```python
from build123d import *

# Parameters (mm, degrees)
SKETCH_1_R      = 17.5
EXTRUDE_1_DEPTH = 31
SKETCH_2_R      = 15
EXTRUDE_2_DEPTH = 43
SKETCH_4_R      = 18.5
EXTRUDE_3_DEPTH = 4


with BuildPart() as part:
    # 草图1 → 凸台-拉伸1 (new body)
    with BuildSketch(Plane(origin=(0, 0, 0), x_dir=(0, 0, -1), z_dir=(1, 0, 0))):
        Circle(SKETCH_1_R)
    extrude(amount=EXTRUDE_1_DEPTH)

    # 草图2 → 凸台-拉伸2 (add)
    with BuildSketch(Plane.ZY):
        with Locations(Location((0, 0, 0), (0, 0, 180))):
            Circle(SKETCH_2_R)
    extrude(amount=EXTRUDE_2_DEPTH)

    # 草图4 → 凸台-拉伸3 (add)
    with BuildSketch(Plane(origin=(12, 0, 0), x_dir=(0, 0, -1), z_dir=(1, 0, 0))):
        Circle(SKETCH_4_R)
    extrude(amount=EXTRUDE_3_DEPTH)


solid = part.part
```
Can you work these out from the model? Positions are in its coordinate system, mm. A direction names the side the tool comes from. Round coordinates to 2 decimals unless told otherwise and drop trailing zeros. Loops run counter-clockwise (first coordinate to the right, second up) from the corner with the lowest first, then second, coordinate; pieces in that order, holes last.
Item 1: Will these pins go through, and if not, where does the flat tip stop? pin 1 Ø3 at (x, z) = (23, -1) entering from +Y; pin 2 Ø5 at (x, z) = (18, -2) entering from -Y; pin 3 Ø1.5 at (x, y) = (12.5, 11.5) entering from +Z; pin 4 Ø8 at (x, y) = (17.5, 1.5) entering from -Z.
Item 2: Which directions (+Z, -Z, +X, -X, +Y, -Y) give clear straight access to the entire face, cutting with the end or side of a thin tool? Please do faces 1 (the cylindrical face through (5.916, -10.648, 13.887)), 2 (the flat face through (16, -14, 11)), 3 (the cylindrical face through (13.97, -18.06, 4.01)).
Item 3: Suppose I cut it at C-C, the plane x = 13. Write out the boundary of the cut face in (y, z).
Item 4: Please list where these lines run through material, in increasing order: L1, parallel to X at y = 9, z = 16; L2, parallel to X at y = 9.5, z = -12; L3, parallel to Y at x = -36, z = -7.5.
Item 5: Suppose I cut it at D-D, the plane x = 24.5. Write out the boundary of the cut face in (y, z).
Item 6: Suppose I cut it at A-A, the plane z = 0. Write out the boundary of the cut face in (x, y).
Reported:
1. pin 1: stops at y = 17.5
1. pin 2: stops at y = -18.49
1. pin 3: stops at z = 15.06
1. pin 4: stops at z = -18.5
2. face 1: -X
2. face 2: +X
2. face 3: +X, -X
3. outline: circle Ø37 at (0, 0)
4. L1: x = 12 to 16
4. L2: x = 0 to 31
4. L3: y = -12.99 to 12.99
5. outline: circle Ø35 at (0, 0)
6. outline: (-43, -15) - (0, -15) - (0, -17.5) - (12, -17.5) - (12, -18.5) - (16, -18.5) - (16, -17.5) - (31, -17.5) - (31, 17.5) - (16, 17.5) - (16, 18.5) - (12, 18.5) - (12, 17.5) - (0, 17.5) - (0, 15) - (-43, 15) - close
